Source: CAD feature listing. Evaluate the final solid. Frame: model axes, mm. Give positions to 0.01 mm unless a question says otherwise; leave off trailing zeros. Loops run counter-clockwise (first coordinate to the right, second up) from the corner with the lowest first, then second, coordinate; pieces in that order, holes last. Notation, with made-up numbers: M -11,31 L 19,31 A23 cw 19,45 Z; hole C -22.5,60.5 d9. An arc over 180 degrees is marked long. Write item = value, one per line.
from build123d import *

# Parameters (mm, degrees)
SKETCH1_W                  = 130
SKETCH1_H                  = 130
BOSS_EXTRUDE1_DEPTH        = 8
F_14_0_14_DIAMETER_HOLE1_D = 14


with BuildPart() as part:
    # Sketch1 → Boss-Extrude1 (new body)
    with BuildSketch(Plane(origin=(0, 0, 0), x_dir=(1, 0, 0), z_dir=(0, 1, 0))):
        Rectangle(SKETCH1_W, SKETCH1_H)
    extrude(amount=BOSS_EXTRUDE1_DEPTH)

    # Ø14.0 (14) Diameter Hole1 (through all)
    with Locations(Plane(origin=(0, 8, 0), x_dir=(1, 0, 0), z_dir=(0, 1, 0))):
        with Locations((-50, -50), (50, -50), (50, 50), (-50, 50)):
            Hole(F_14_0_14_DIAMETER_HOLE1_D / 2)


solid = part.part
1. Cut plane C-C, the plane y = 2. Return the cut outline in (x, z), then the cut area to 3 significant figures.
Derived:
outline = M -65,-65 L 65,-65 L 65,65 L -65,65 Z; hole C -50,-50 d14; hole C -50,50 d14; hole C 50,-50 d14; hole C 50,50 d14
area = 16,300 mm²
2. Pull-direction query (Z, two-part tool) for faces 1 (the flat face through (-1, 8, -1)), 2 (the flat face through (-1, 4, -65)), 3 (the cylindrical face through (43.323, 3.944, -52.103)); classes: +Z half, -Z half, draft (parallel to the pull), parting line (faces both ways), or undercut.
Derived:
face_1 = draft
face_2 = -Z half
face_3 = undercut
3. Cut plane A-A, the plane z = 50. Return the cut outline in (x, y), then the cut area to 3 significant figures.
Derived:
outline = M -65,0 L -57,0 L -57,8 L -65,8 Z; M -43,0 L 43,0 L 43,8 L -43,8 Z; M 57,0 L 65,0 L 65,8 L 57,8 Z
area = 816 mm²
4. Material intervals for probe 1 along Z at (x, y) = (-50, 3.5); probe 2 along Z at (x, y) = (56, 6.75), sorted ascending. Write a range as from..to.
Derived:
probe_1 = -65..-57, -43..43, 57..65
probe_2 = -65..-53.61, -46.39..46.39, 53.61..65
5. Cut plane B-B, the plane x = -50. Return the cut outline in (y, z).
Derived:
outline = M 0,-65 L 8,-65 L 8,-57 L 0,-57 Z; M 0,-43 L 8,-43 L 8,43 L 0,43 Z; M 0,57 L 8,57 L 8,65 L 0,65 Z
